```python
from build123d import *

# Parameters (mm, degrees)
BOSS_EXTRUDE1_DEPTH   = 10
M5_TAPPED_HOLE1_D     = 4.2
M5_TAPPED_HOLE1_DEPTH = 14
M5_TAPPED_HOLE1_TIP   = 1.2618073
M5_TAPPED_HOLE2_D     = 4.2
M5_TAPPED_HOLE2_DEPTH = 14
M5_TAPPED_HOLE2_TIP   = 1.2618073


with BuildPart() as part:
    # Sketch1 → Boss-Extrude1 (new body)
    with BuildSketch(Plane.XY):
        Polygon((0, 0), (-320, 42), (-320, 47), (0, 47), align=None)
    extrude(amount=BOSS_EXTRUDE1_DEPTH)

    # M5 Tapped Hole1
    with Locations(Plane(origin=(0, 47, 0), x_dir=(-1, 0, 0), z_dir=(0, 1, 0))):
        with Locations((287.5, 5), (202.5, 5), (117.5, 5), (32.5, 5)):
            Hole(M5_TAPPED_HOLE1_D / 2, depth=M5_TAPPED_HOLE1_DEPTH)
            with Locations((0, 0, -(M5_TAPPED_HOLE1_DEPTH + M5_TAPPED_HOLE1_TIP / 2))):  # 118° drill point
                Cone(0, M5_TAPPED_HOLE1_D / 2, M5_TAPPED_HOLE1_TIP, mode=Mode.SUBTRACT)

    # M5 Tapped Hole2
    with Locations(Plane(origin=(0, 0, 0), x_dir=(0, 0, -1), z_dir=(1, 0, 0))):
        with Locations((-5, 41), (-5, 25), (-5, 9)):
            Hole(M5_TAPPED_HOLE2_D / 2, depth=M5_TAPPED_HOLE2_DEPTH)
            with Locations((0, 0, -(M5_TAPPED_HOLE2_DEPTH + M5_TAPPED_HOLE2_TIP / 2))):  # 118° drill point
                Cone(0, M5_TAPPED_HOLE2_D / 2, M5_TAPPED_HOLE2_TIP, mode=Mode.SUBTRACT)


solid = part.part
```
Could you check a few things on this model? Use its own coordinates, in mm. Coordinates: 2 decimals unless noted, no trailing zeros. Write each loop counter-clockwise with the first axis right and the second up, starting at its lowest first coordinate (ties: lowest second). Pieces come first, ordered by that corner, then holes. Notation, with made-up numbers: (1.5, 83.25) -> (23.5, 83.25) arc R17 cw to (23.5, 110.25) -> close; hole circle Ø7 at (-17, 62.5). An arc over 180 degrees is marked (long way). One line per question, with ' | ' between items. Start each with the question number.
1. If we section it at B-B (x = -156.5): Please give me the cut outline in (y, z), and give its area (3 significant figures).
2. Will these pins go through, and if not, where does the flat tip stop? P1, Ø4, axis at x = -202.5, z = 5, coming from the -Y side; P2, Ø3, axis at x = -125.5, z = 2.5, coming from the -Y side (3 decimals); P3, Ø4, axis at x = -32.5, z = 5, coming from the -Y side.
3. If we section it at A-A (x = -52.5): Please give me the cut outline in (y, z), and give its area (3 significant figures).
4. Please list where these lines run through material, in increasing order: line 1 along X through (y, z) = (37.5, 5); line 2 along Z through (x, y) = (-9.25, 9); line 3 along Z through (x, y) = (-117, 39).
Return value:
1) outline: (20.54, 0) -> (47, 0) -> (47, 10) -> (20.54, 10) -> close | area: 265 mm²
2) P1: stops at y = 26.32 | P2: stops at y = 16.275 | P3: stops at y = 4
3) outline: (6.89, 0) -> (47, 0) -> (47, 10) -> (6.89, 10) -> close | area: 401 mm²
4) line 1: x = -285.4 to -204.6, -200.4 to -119.6, -115.4 to -34.6, -30.4 to 0 | line 2: z = 0 to 2.9, 7.1 to 10 | line 3: z = 0 to 2.96, 7.04 to 10
